CAD build for the part. Positions are in the model's coordinates, mm. A direction names the side the tool comes from. Round coordinates to 2 decimals unless told otherwise and drop trailing zeros. Loops run counter-clockwise (first coordinate to the right, second up) from the corner with the lowest first, then second, coordinate; pieces in that order, holes last. Notation, with made-up numbers: M 6.5,-13 L 49.5,-13 A22 cw 49.5,24 Z; hole C -9,40.5 d8. An arc over 180 degrees is marked long. Use a Markdown table: item, result. Add a question column.
(1) Flat gauge pins, fed straight in: P1, Ø5, axis at x = -7.5, z = 33, coming from the +Y side; P2, Ø1.5, axis at y = -26, z = 78, coming from the +X side; P3, Ø8, axis at x = -13.5, y = 14.5, coming from the +Z side. Where does each tip first touch, or does it go through?
(2) Band-saw the part on B-B, the plane z = 107. Write the cut outline in (x, y).
(3) Band-saw the part on C-C, the plane x = 0. Write the cut outline in (y, z).
(4) Wall check: L1, parallel to Z at x = 23, y = -28; L2, parallel to Y at x = -22.5, z = 122.5; L3, parallel to Z at x = 2, y = -14. Give the ranges that are in metal, low to high.
(5) Which spindle directions (+Z, -Z, +X, -X, +Y, -Y) get a long thin tool onto all of the face, cutting with end or side? Do faces 5 (the face through (27, -27, 135.5)), 6 (the face through (-4.336, -19.524, 45.28)), 7 (the face through (0, -32.5, 127)). Say none if no direction does.
(6) Band-saw the part on D-D, the plane z = 127.5. Write the cut outline in (x, y), and give its area (3 significant figures).
(7) Two-plate mould, pull along Y, no slides. Class faces 1 (the face through (40.634, 0.308, 134.493)), 2 (the face through (36.86, -21.16, 12.32)), 3 (the face through (25.488, 21.577, 137.782)), 4 (the face through (22.97, -22.85, 125.39)): released by +Y, released by -Y, zero draft, split by the parting line, or undercut.
(8) Band-saw the part on A-A, the plane x = 44.5. Write the cut outline in (y, z), and give its area (3 significant figures).
from build123d import *

# Parameters (mm, degrees)
HEX_BODY_DEPTH                     = 25
BODY_PROFILE_60_R                  = 30
BODY_CYLINDER_60_DEPTH             = 90
SQUARE_FLANGE_DEPTH                = 25
FLANGE_BORE_PROFILE_50_R           = 25
FLANGE_BORE_50_DEPTH               = 25
THROUGH_BORE_PROFILE_20_R          = 10
THROUGH_BORE_20_DEPTH              = 50
HEX_END_BORE_PROFILE_40_R          = 20
HEX_END_BORE_40_DEPTH              = 40
HEX_EDGE_FILLET_R5_A_R             = 5
HEX_EDGE_FILLET_R5_B_R             = 5
HEX_EDGE_FILLET_R5_C_R             = 5
HEX_EDGE_FILLET_R5_D_R             = 5
HEX_EDGE_FILLET_R5_E_R             = 5
HEX_EDGE_FILLET_R5_F_R             = 5
COUNTERBORE_PROFILE_4X_7_5_R       = 3.75
MOUNTING_COUNTERBORES_4X_7_5_DEPTH = 4.5
MOUNTING_HOLE_PROFILE_4X_5_5_R     = 2.75
MOUNTING_HOLES_4X_5_5_DEPTH        = 20.5
PORT_BOSS_PROFILE_14_R             = 7
PRESSURE_PORT_BOSS_14_DEPTH        = 17.5
PORT_BOSS_TIP_FILLET_R1_R          = 1
PORT_HOLE_PROFILE_5_R              = 2.5
PORT_HOLE_5_DEPTH                  = 28
BODY_TO_HEX_FILLET_R2_R            = 2


with BuildPart() as part:
    # Hex Profile → Hex Body (new body)
    with BuildSketch(Plane.XY):
        Polygon((24.12843754, 42.733497812), (-24.944075927, 42.262588769), (-49.072513467, -0.470909043), (-24.12843754, -42.733497812), (24.944075927, -42.262588769), (49.072513467, 0.470909043), align=None)
    extrude(amount=HEX_BODY_DEPTH)

    # Body Profile Ø60 → Body Cylinder Ø60 (add)
    with BuildSketch(Plane.XY.offset(25)):
        with Locations(Location((0, 0, 0), (0, 0, 180))):
            Circle(BODY_PROFILE_60_R)
    extrude(amount=BODY_CYLINDER_60_DEPTH)

    # Flange Profile 65x65 → Square Flange (add)
    with BuildSketch(Plane.XY.offset(115)):
        with BuildLine():
            Line((-22.5, -32.5), (22.5, -32.5))
            ThreePointArc((22.5, -32.5), (29.571067812, -29.571067812), (32.5, -22.5))
            Line((32.5, -22.5), (32.5, 22.5))
            ThreePointArc((32.5, 22.5), (29.571067812, 29.571067812), (22.5, 32.5))
            Line((22.5, 32.5), (-22.5, 32.5))
            ThreePointArc((-22.5, 32.5), (-29.571067812, 29.571067812), (-32.5, 22.5))
            Line((-32.5, 22.5), (-32.5, -22.5))
            ThreePointArc((-32.5, -22.5), (-29.571067812, -29.571067812), (-22.5, -32.5))
        make_face()
    extrude(amount=SQUARE_FLANGE_DEPTH)

    # Flange Bore Profile Ø50 → Flange Bore Ø50 (cut)
    with BuildSketch(Plane.XY.offset(140)):
        Circle(FLANGE_BORE_PROFILE_50_R)
    extrude(amount=-FLANGE_BORE_50_DEPTH, mode=Mode.SUBTRACT)

    # Through Bore Profile Ø20 → Through Bore Ø20 (cut)
    with BuildSketch(Plane.XY.offset(115)):
        Circle(THROUGH_BORE_PROFILE_20_R)
    extrude(amount=-THROUGH_BORE_20_DEPTH, mode=Mode.SUBTRACT)

    # Hex End Bore Profile Ø40 → Hex End Bore Ø40 (cut)
    with BuildSketch(Plane.XY.offset(65)):
        Circle(HEX_END_BORE_PROFILE_40_R)
    extrude(amount=-HEX_END_BORE_40_DEPTH, mode=Mode.SUBTRACT)

    # Hex Edge Fillet R5 A
    hex_edge_fillet_r5_a_edges = [part.edges().sort_by_distance(p)[0] for p in [
        (24.12843754, 42.733497812, 12.5),
    ]]
    fillet(hex_edge_fillet_r5_a_edges, radius=HEX_EDGE_FILLET_R5_A_R)

    # Hex Edge Fillet R5 B
    hex_edge_fillet_r5_b_edges = [part.edges().sort_by_distance(p)[0] for p in [
        (49.072513467, 0.470909043, 12.5),
    ]]
    fillet(hex_edge_fillet_r5_b_edges, radius=HEX_EDGE_FILLET_R5_B_R)

    # Hex Edge Fillet R5 C
    hex_edge_fillet_r5_c_edges = [part.edges().sort_by_distance(p)[0] for p in [
        (-24.944075927, 42.262588769, 12.5),
    ]]
    fillet(hex_edge_fillet_r5_c_edges, radius=HEX_EDGE_FILLET_R5_C_R)

    # Hex Edge Fillet R5 D
    hex_edge_fillet_r5_d_edges = [part.edges().sort_by_distance(p)[0] for p in [
        (-49.072513467, -0.470909043, 12.5),
    ]]
    fillet(hex_edge_fillet_r5_d_edges, radius=HEX_EDGE_FILLET_R5_D_R)

    # Hex Edge Fillet R5 E
    hex_edge_fillet_r5_e_edges = [part.edges().sort_by_distance(p)[0] for p in [
        (-24.12843754, -42.733497812, 12.5),
    ]]
    fillet(hex_edge_fillet_r5_e_edges, radius=HEX_EDGE_FILLET_R5_E_R)

    # Hex Edge Fillet R5 F
    hex_edge_fillet_r5_f_edges = [part.edges().sort_by_distance(p)[0] for p in [
        (24.944075927, -42.262588769, 12.5),
    ]]
    fillet(hex_edge_fillet_r5_f_edges, radius=HEX_EDGE_FILLET_R5_F_R)

    # Counterbore Profile 4xØ7.5 → Mounting Counterbores 4xØ7.5 (cut)
    with BuildSketch(Plane.XY.offset(140)):
        with Locations((-25, 25.295084972)):
            Circle(COUNTERBORE_PROFILE_4X_7_5_R)
        with Locations((-25, -24.704915028)):
            Circle(COUNTERBORE_PROFILE_4X_7_5_R)
        with Locations(Location((25, -24.704915028, 0), (0, 0, 180))):
            Circle(COUNTERBORE_PROFILE_4X_7_5_R)
        with Locations(Location((25, 25.295084972, 0), (0, 0, 180))):
            Circle(COUNTERBORE_PROFILE_4X_7_5_R)
    extrude(amount=-MOUNTING_COUNTERBORES_4X_7_5_DEPTH, mode=Mode.SUBTRACT)

    # Mounting Hole Profile 4xØ5.5 → Mounting Holes 4xØ5.5 (cut)
    with BuildSketch(Plane.XY.offset(135.5)):
        with Locations((-25, 25.295084972)):
            Circle(MOUNTING_HOLE_PROFILE_4X_5_5_R)
        with Locations((25, 25.295084972)):
            Circle(MOUNTING_HOLE_PROFILE_4X_5_5_R)
        with Locations((25, -24.704915028)):
            Circle(MOUNTING_HOLE_PROFILE_4X_5_5_R)
        with Locations((-25, -24.704915028)):
            Circle(MOUNTING_HOLE_PROFILE_4X_5_5_R)
    extrude(amount=-MOUNTING_HOLES_4X_5_5_DEPTH, mode=Mode.SUBTRACT)

    # Port Boss Profile Ø14 → Pressure Port Boss Ø14 (add)
    with BuildSketch(Plane(origin=(32.5, 0, 0), x_dir=(0, 0, -1), z_dir=(1, 0, 0))):
        with Locations((-127.5, 0)):
            Circle(PORT_BOSS_PROFILE_14_R)
    extrude(amount=PRESSURE_PORT_BOSS_14_DEPTH)

    # Port Boss Tip Fillet R1
    port_boss_tip_fillet_r1_edges = [part.edges().sort_by_distance(p)[0] for p in [
        (50, 0, 134.5),
    ]]
    fillet(port_boss_tip_fillet_r1_edges, radius=PORT_BOSS_TIP_FILLET_R1_R)

    # Port Hole Profile Ø5 → Port Hole Ø5 (cut)
    with BuildSketch(Plane(origin=(50, 0, 0), x_dir=(0, 0, -1), z_dir=(1, 0, 0))):
        with Locations((-127.5, 0)):
            Circle(PORT_HOLE_PROFILE_5_R)
    extrude(amount=-PORT_HOLE_5_DEPTH, mode=Mode.SUBTRACT)

    # Body to Hex Fillet R2
    body_to_hex_fillet_r2_edges = [part.edges().sort_by_distance(p)[0] for p in [
        (30, 0, 25),
    ]]
    fillet(body_to_hex_fillet_r2_edges, radius=BODY_TO_HEX_FILLET_R2_R)


solid = part.part
Return value:
| question | item | result |
|---|---|---|
| 1 | P1 | y = 29.58 |
| 1 | P2 | x = 16.2 |
| 1 | P3 | z = 115 |
| 2 | outline | C 0,0 d60; hole C 0,0 d20 |
| 3 | outline | M -42.5,0 L 42.5,0 L 42.5,25 L 32,25 A2 cw 30,27 L 30,115 L 32.5,115 L 32.5,140 L 25,140 L 25,115 L 10,115 L 10,65 L 20,65 L 20,25 L -20,25 L -20,65 L -10,65 L -10,115 L -25,115 L -25,140 L -32.5,140 L -32.5,115 L -30,115 L -30,27 A2 cw -32,25 L -42.5,25 Z |
| 4 | L1 | 0 to 25, 115 to 140 |
| 4 | L2 | -32.5 to -25.85, -23.56 to -10.9, 10.9 to 24.15, 26.44 to 32.5 |
| 4 | L3 | 0 to 25, 65 to 115 |
| 5 | face 5 | +Z |
| 5 | face 6 | none |
| 5 | face 7 | +Z, +X, -X, -Y |
| 6 | outline | M -32.5,-22.5 A10 ccw -22.5,-32.5 L 22.5,-32.5 A10 ccw 32.5,-22.5 L 32.5,-7 L 49,-7 A1 ccw 50,-6 L 50,-2.5 L 24.87,-2.5 A25 cw long 24.87,2.5 L 50,2.5 L 50,6 A1 ccw 49,7 L 32.5,7 L 32.5,22.5 A10 ccw 22.5,32.5 L -22.5,32.5 A10 ccw -32.5,22.5 Z; hole C -25,-24.7 d5.5; hole C -25,25.3 d5.5; hole C 25,-24.7 d5.5; hole C 25,25.3 d5.5 |
| 6 | area | 2,200 mm^2 |
| 7 | face 1 | split by the parting line |
| 7 | face 2 | released by -Y |
| 7 | face 3 | undercut |
| 7 | face 4 | undercut |
| 8 | outline | M -7.63,0 L 8.22,0 L 8.22,25 L -7.63,25 Z; C 0,127.5 d14; hole C 0,127.5 d5 |
| 8 | area | 530 mm^2 |
